Part model, mm, in its own coordinate system. A direction names the side the tool comes from. Round coordinates to 2 decimals unless told otherwise and drop trailing zeros. Loops run counter-clockwise (first coordinate to the right, second up) from the corner with the lowest first, then second, coordinate; pieces in that order, holes last.
1) Probe line 1 (Y direction, x = 44, z = 0); line 2 (X direction, y = -27, z = -12.25); line 3 (Z direction, x = 86.5, y = 1). List the from-to ranges inside material, lowest first.
2) 3-axis set-ups, long thin cutter, end or side, ignore diameter. For faces 1 (the cylindrical face through (123.03, -4.38, 14.74)), 2 (the cylindrical face through (13.79, -25.09, -10.84)), 3 (the flat face through (66, -15, 12)), 4 (the flat face through (66, -25, 15)): which of +Z, -Z, +X, -X, +Y, -Y reach the whole face in a straight line?
3) Band-saw the part on B-B, the plane x = 85. State how many separate pieces and enclosed holes the cut face has, then the cut area to 3 significant figures.
4) Band-saw the part on A-A, the plane z = 0. Write the cut outline in (x, y), then the cut area to 3 significant figures.
5) Mould opens along Y. For faces 5 (the flat face through (66, 32, 12)), 6 (the flat face through (66, 25, 15)), 7 (the cylindrical face through (126.37, 19.6, -9.48)) say: +Y half, -Y half, draft (parallel to the pull), parting line (faces both ways), or undercut.
6) Drop flat-ended pins along their axis: P1, Ø1.4, axis at x = 33.5, y = -13.5, coming from the +Z side; P2, Ø1, axis at y = -1.5, z = -6, coming from the -X side; P3, Ø3.5, axis at x = 11.5, y = -4.5, coming from the +Z side; P4, Ø0.6, axis at x = 97, y = 1, coming from the -Z side. Give the stop position or say it passes through.
from build123d import *

# Parameters (mm, degrees)
SKETCH_1_W                  = 33
SKETCH_1_H                  = 64
EXTRUDE_1_DEPTH             = 133
HOLE_WIZARD_1_D             = 10
PATTERN_LINEAR_1_COUNT      = 2
PATTERN_LINEAR_1_PITCH      = 38
PATTERN_LINEAR_2_COUNT      = 2
PATTERN_LINEAR_2_PITCH      = 22
PATTERN_LINEAR_2_COUNT_DIR2 = 2
PATTERN_LINEAR_2_PITCH_DIR2 = 42
PATTERN_LINEAR_3_COUNT      = 2
PATTERN_LINEAR_3_PITCH      = 107
PATTERN_LINEAR_3_COUNT_DIR2 = 2
PATTERN_LINEAR_3_PITCH_DIR2 = 54
CUT_EXTRUDE_1_DEPTH         = 133
CUT_EXTRUDE_2_DEPTH         = 133
CUT_EXTRUDE_3_DEPTH         = 133
CUT_EXTRUDE_4_DEPTH         = 133
CUT_EXTRUDE_5_DEPTH         = 133
HOLE_WIZARD_4_D             = 4.134
HOLE_WIZARD_4_DEPTH         = 6
HOLE_WIZARD_4_CSINK_D       = 5
HOLE_WIZARD_4_CSINK_ANGLE   = 90
PATTERN_LINEAR_4_COUNT      = 2
PATTERN_LINEAR_4_PITCH      = 114


with BuildPart() as part:
    # 草图1 → 凸台-拉伸1 (new body)
    with BuildSketch(Plane(origin=(0, 0, 0), x_dir=(0, 0, -1), z_dir=(1, 0, 0))):
        with Locations((-1.5, 0)):
            Rectangle(SKETCH_1_W, SKETCH_1_H)
    extrude(amount=EXTRUDE_1_DEPTH)

    # 孔1 (through all)
    with Locations(Plane(origin=(133, 0, 0), x_dir=(0, 0, -1), z_dir=(1, 0, 0))):
        with Locations((0, 19)):
            hole_wizard_1 = Hole(HOLE_WIZARD_1_D / 2)

    # 阵列(线性)1: 孔1 ×2
    with Locations(*[(0, -i * PATTERN_LINEAR_1_PITCH, 0) for i in range(1, PATTERN_LINEAR_1_COUNT)]):
        add(hole_wizard_1, mode=Mode.SUBTRACT)

    # 草图5 → 孔2 (revolve, cut)
    with BuildSketch(Plane(origin=(133, 21, 11), x_dir=(0, 0, -1), z_dir=(0, 1, 0))):
        Polygon((0, 0), (0, 14.099043395), (2.067, 13), (2.067, 0.433), (2.5, 0), align=None)
    hole_wizard_2 = revolve(axis=Axis((147.308894879, 21, 11), (-1, 0, 0)), mode=Mode.SUBTRACT)

    # 阵列(线性)2: Hole Wizard 2 2 × 2
    with Locations(*[(0, -j * PATTERN_LINEAR_2_PITCH_DIR2, -i * PATTERN_LINEAR_2_PITCH) for i in range(PATTERN_LINEAR_2_COUNT) for j in range(PATTERN_LINEAR_2_COUNT_DIR2) if (i, j) != (0, 0)]):
        add(hole_wizard_2, mode=Mode.SUBTRACT)

    # 草图8 → 孔3 (revolve, cut)
    with BuildSketch(Plane(origin=(13, 27, -15), x_dir=(0, 1, 0), z_dir=(1, 0, 0))):
        Polygon((0, 0), (0, 9.099043395), (2.067, 8), (2.067, 0.433), (2.5, 0), align=None)
    hole_wizard_3 = revolve(axis=Axis((13, 27, -29.308894879), (0, 0, 1)), mode=Mode.SUBTRACT)

    # 阵列(线性)3: Hole Wizard 3 2 × 2
    with Locations(*[(i * PATTERN_LINEAR_3_PITCH, -j * PATTERN_LINEAR_3_PITCH_DIR2, 0) for i in range(PATTERN_LINEAR_3_COUNT) for j in range(PATTERN_LINEAR_3_COUNT_DIR2) if (i, j) != (0, 0)]):
        add(hole_wizard_3, mode=Mode.SUBTRACT)

    # 草图11 → 切除-旋转1 (revolve, cut)
    with BuildSketch(Plane.XY, mode=Mode.PRIVATE) as cut_revolve_1_sk:
        Polygon((0, 0), (0, 4), (16.5, 4), (16.5, 8), (121.5, 8), (121.5, 0), align=None)
    revolve(cut_revolve_1_sk.sketch.rotate(Axis((121.5, 0, 0), (-1, 0, 0)), 270), axis=Axis((121.5, 0, 0), (-1, 0, 0)), mode=Mode.SUBTRACT)

    # 草图12 → 切除-拉伸1 (cut)
    with BuildSketch(Plane(origin=(0, 0, 0), x_dir=(0, 0, -1), z_dir=(1, 0, 0))):
        with BuildLine():
            Line((-8, 32), (-4.865738712, 26.571300205))
            ThreePointArc((-4.865738712, 26.571300205), (-0.867061595, 27.958136201), (3.323361728, 27.36392652))
            Line((3.323361728, 27.36392652), (6, 32))
            Line((6, 32), (-8, 32))
        make_face()
    extrude(amount=CUT_EXTRUDE_1_DEPTH, mode=Mode.SUBTRACT)

    # 草图13 → 切除-拉伸2 (cut)
    with BuildSketch(Plane(origin=(0, 0, 0), x_dir=(0, 0, -1), z_dir=(1, 0, 0))):
        with BuildLine():
            Line((-8, -32), (6, -32))
            Line((6, -32), (3.323361728, -27.36392652))
            ThreePointArc((3.323361728, -27.36392652), (-0.867061595, -27.958136201), (-4.865738712, -26.571300205))
            Line((-4.865738712, -26.571300205), (-8, -32))
        make_face()
    extrude(amount=CUT_EXTRUDE_2_DEPTH, mode=Mode.SUBTRACT)

    # 草图14 → 切除-拉伸3 (cut)
    with BuildSketch(Plane(origin=(0, 0, 0), x_dir=(0, 0, -1), z_dir=(1, 0, 0))):
        with BuildLine():
            Line((7.5, -12), (15, -19.5))
            Line((15, -19.5), (15, 19.5))
            Line((15, 19.5), (7.5, 12))
            Line((7.5, 12), (7.5, 8.717797887))
            ThreePointArc((7.5, 8.717797887), (11.5, 0), (7.5, -8.717797887))
            Line((7.5, -8.717797887), (7.5, -12))
        make_face()
    extrude(amount=CUT_EXTRUDE_3_DEPTH, mode=Mode.SUBTRACT)

    # 草图15 → 切除-拉伸4 (cut)
    with BuildSketch(Plane(origin=(0, 0, 0), x_dir=(0, 0, -1), z_dir=(1, 0, 0))):
        Polygon((-18, -32), (-15, -32), (-15, -18.5), (-12, -16.767949192), (-12, -12.183821406), (-18, -10), align=None)
    extrude(amount=CUT_EXTRUDE_4_DEPTH, mode=Mode.SUBTRACT)

    # 草图16 → 切除-拉伸5 (cut)
    with BuildSketch(Plane(origin=(0, 0, 0), x_dir=(0, 0, -1), z_dir=(1, 0, 0))):
        Polygon((-18, 32), (-18, 0.8235), (-17.4691, 1.743045774), (-16.655766975, 1.273467733), (-16.655766975, 0.551779896), (-13.451472981, -1.298220104), (-10.301472981, 4.15773994), (-13.505766975, 6.00773994), (-14.130766975, 5.646896022), (-14.9441, 6.116474063), (-12.76915, 9.883597967), (-11.955816975, 9.414019926), (-11.955816975, 8.692332089), (-8.751522981, 6.842332089), (-5.601522981, 12.298292133), (-8.805816975, 14.148292133), (-9.430816975, 13.787448215), (-11, 14.693416457), (-11, 16.190598923), (-15, 18.5), (-15, 32), align=None)
    extrude(amount=CUT_EXTRUDE_5_DEPTH, mode=Mode.SUBTRACT)

    # 孔4
    with Locations(Plane.XY.offset(18)):
        with Locations((11, -5)):
            hole_wizard_4 = CounterSinkHole(HOLE_WIZARD_4_D / 2, HOLE_WIZARD_4_CSINK_D / 2, depth=HOLE_WIZARD_4_DEPTH, counter_sink_angle=HOLE_WIZARD_4_CSINK_ANGLE)

    # 阵列(线性)4: 孔4 ×2
    with Locations(*[(i * PATTERN_LINEAR_4_PITCH, 0, 0) for i in range(1, PATTERN_LINEAR_4_COUNT)]):
        add(hole_wizard_4, mode=Mode.SUBTRACT)


solid = part.part
Reported:
1. line 1: y = -28 to -24, -14 to -8, 8 to 14, 24 to 28
1. line 2: x = 0 to 10.93, 15.07 to 117.93, 122.07 to 133
1. line 3: z = -11.46 to -7.94, 7.94 to 12.12, 16.66 to 17.9
2. face 1: +Z
2. face 2: -Z
2. face 3: +Z, +X, -X
2. face 4: +Z, +X, -X, -Y
3. separate pieces: 1
3. enclosed holes: 3
3. area: 1,200 mm2
4. outline: (0, -28) - (133, -28) - (133, -24) - (0, -24) - close; (0, -14) - (133, -14) - (133, 14) - (0, 14) - (0, 4) - (16.5, 4) - (16.5, 8) - (121.5, 8) - (121.5, -8) - (16.5, -8) - (16.5, -4) - (0, -4) - close; (0, 24) - (133, 24) - (133, 28) - (0, 28) - close
4. area: 2,980 mm2
5. face 5: +Y half
5. face 6: draft
5. face 7: undercut
6. P1: stops at z = 12
6. P2: stops at x = 0
6. P3: stops at z = 17.96
6. P4: stops at z = -11.48
